from build123d import *

# Parameters (mm, degrees)
SKETCH_1_R      = 16.5
SKETCH_1_R_2    = 7.5
EXTRUDE_1_DEPTH = 10
SKETCH_2_R      = 9
SKETCH_2_R_2    = 7.5
EXTRUDE_2_DEPTH = 1
EXTRUDE_START   = 3
SKETCH_3_R      = 16.5
EXTRUDE_3_DEPTH = 3
CHAMFER_1_SIZE  = 2


with BuildPart() as part:
    # 草图1 → 凸台-拉伸1 (new body)
    with BuildSketch(Plane.XY):
        Circle(SKETCH_1_R)
        Circle(SKETCH_1_R_2, mode=Mode.SUBTRACT)
    extrude(amount=EXTRUDE_1_DEPTH)

    # 草图2 → 凸台-拉伸2 (add)
    with BuildSketch(Plane.XY.offset(10)):
        Circle(SKETCH_2_R)
        Circle(SKETCH_2_R_2, mode=Mode.SUBTRACT)
    extrude(amount=EXTRUDE_2_DEPTH)

    # 草图3 → 凸台-拉伸3 (add)
    with BuildSketch(Plane(origin=(0, 0, 0), x_dir=(-1, 0, 0), z_dir=(0, 0, -1)).offset(EXTRUDE_START)):
        Circle(SKETCH_3_R)
    extrude(amount=-EXTRUDE_3_DEPTH)

    # 倒角1
    chamfer_1_edges = [part.edges().sort_by_distance(p)[0] for p in [
        (16.5, 0, -3),
        (-16.5, 0, 10),
    ]]
    chamfer(chamfer_1_edges, length=CHAMFER_1_SIZE)


solid = part.part
Read the model definition and answer for the solid it produces. Units are mm, in the model's axes. A direction names the side the tool comes from. Round coordinates to 2 decimals unless told otherwise and drop trailing zeros. Order: outer loops, then holes, each group sorted by start corner. A loop starts at its lowest first (then second) coordinate and runs counter-clockwise, first axis right, second up.
1) The part is cut by section A-A on y = 0. Write down the section's boundary in (x, z), plus the area to 3 significant figures.
2) Flat-ended cylindrical pins translate along their axes: pin 1 (1.5 mm diameter, centred on x = 6, z = 3, fed in from +Y); pin 2 (4 mm diameter, centred on x = -2.5, z = 7.5, fed in from +Y); pin 3 (1.5 mm diameter, centred on x = -1.5, y = -12, fed in from +Z). Find the tip coordinate at first contact, or state that the pin passes through.
3) For faces 1 (the face through (0, 0, 0)), 2 (the face through (0, 0, -3)), determine the directions among +Z, -Z, +X, -X, +Y, -Y from which every point of the face is accessible in a straight line to the end or side of a thin tool.
4) The mould has two halves that part along X. Classify faces 3 (the face through (-1.172, 8.923, 10.493)), 4 (the face through (-7.493, 0.33, 5.423)), 5 (the face through (-2, 7.4, 11)): released by +X, released by -X, zero draft, split by the parting line, or undercut.
5) Straight lines are drawn through the part: L1, parallel to Y at x = 0, z = 7; L2, parallel to Z at x = 10, y = 4; L3, parallel to Y at x = 0, z = 8.75. For each, find the intervals that lie inside material, in ascending order.
6) The part is cut by section C-C on z = 1.5. Write down the section's boundary in (x, y).
Resolved:
1. outline: (-16.5, -1) - (-14.5, -3) - (14.5, -3) - (16.5, -1) - (16.5, 8) - (14.5, 10) - (9, 10) - (9, 11) - (7.5, 11) - (7.5, 0) - (-7.5, 0) - (-7.5, 11) - (-9, 11) - (-9, 10) - (-14.5, 10) - (-16.5, 8) - close
1. area: 274 mm2
2. pin 1: stops at y = 15.64
2. pin 2: stops at y = 16.49
2. pin 3: stops at z = 10
3. face 1: +Z
3. face 2: -Z, +X, -X, +Y, -Y
4. face 3: split by the parting line
4. face 4: undercut
4. face 5: zero draft
5. L1: y = -16.5 to -7.5, 7.5 to 16.5
5. L2: z = -3 to 10
5. L3: y = -15.75 to -7.5, 7.5 to 15.75
6. outline: circle Ø33 at (0, 0); hole circle Ø15 at (0, 0)
